```python
from build123d import *


with BuildPart() as part:
    # 草图1 → 旋转1 (revolve)
    with BuildSketch(Plane.XY, mode=Mode.PRIVATE) as revolve_1_sk:
        Polygon((20, 9.76740105), (20, -50.23259895), (51.5, -50.23259895), (51.5, -44.23259895), (57.5, -44.23259895), (57.5, 3.76740105), (51.5, 3.76740105), (51.5, 9.76740105), align=None)
    revolve(revolve_1_sk.sketch.rotate(Axis((0, 27.589183228, 0), (0, -1, 0)), 90), axis=Axis((0, 27.589183228, 0), (0, -1, 0)))


solid = part.part
```
Geometry check sheet. Reference: the model listing, model coordinates, mm. A direction names the side the tool comes from. Round coordinates to 2 decimals unless told otherwise and drop trailing zeros. Order: outer loops, then holes, each group sorted by start corner. A loop starts at its lowest first (then second) coordinate and runs counter-clockwise, first axis right, second up. Notation, with made-up numbers: (58, 56.25) - (77, 56.25) arc R28 cw to (77, 78.25) - close; hole circle Ø8 at (30, 7). An arc over 180 degrees is marked (long way). Use a Markdown table: item, result. Add a question column.
1) Thickness scan on line 1 along X through (y, z) = (-14, 0); line 2 along Y through (x, z) = (-38.5, 38.5); line 3 along Z through (x, y) = (-3, -26). Record the ranges inside material, lowest first.
2) Section check D-D (x = 40.5). Record the cut outline in (y, z), then the cut area to 3 significant figures.
3) Section check A-A (x = 0). Record the cut outline in (y, z).
4) Section check B-B (z = 5). Record the cut outline in (x, y), then the cut area to 3 significant figures.
5) Set-up check for faces 1 (the flat face through (-1, -50.233, -22)), 2 (the flat face through (30, 3.767, -43)): record each of +Z, -Z, +X, -X, +Y, -Y from which the full face is reachable in a straight line by a thin tool's end or side.
6) Mould release check, pull along Z, two halves, no side actions. Record for faces 3 (the cylindrical face through (50.275, -47.191, -11.164)), 4 (the flat face through (30, -44.233, 43)), 5 (the cylindrical face through (-0.88, -20.65, -19.98)): released by +Z, released by -Z, zero draft, split by the parting line, or undercut.
7) Section check C-C (y = -24). Record the cut outline in (x, z), then the cut area to 3 significant figures.
8) Gauge pin test, flat ends, axial feed: P1, Ø5, axis at y = 1.5, z = -5.5, coming from the -X side; P2, Ø2, axis at x = -32, y = -9, coming from the +Z side; P3, Ø5, axis at y = -5, z = -35.5, coming from the -X side. Record the tip position at first contact, or that the pin passes through.
Established:
| question | item | result |
|---|---|---|
| 1 | line 1 | -57.5 to -20, 20 to 57.5 |
| 1 | line 2 | -44.23 to 3.77 |
| 1 | line 3 | -57.42 to -19.77, 19.77 to 57.42 |
| 2 | outline | (-50.23, -31.81) - (-44.23, -31.81) - (-44.23, -40.82) - (3.77, -40.82) - (3.77, -31.81) - (9.77, -31.81) - (9.77, 31.81) - (3.77, 31.81) - (3.77, 40.82) - (-44.23, 40.82) - (-44.23, 31.81) - (-50.23, 31.81) - close |
| 2 | area | 4,680 mm2 |
| 3 | outline | (-50.23, -51.5) - (-44.23, -51.5) - (-44.23, -57.5) - (3.77, -57.5) - (3.77, -51.5) - (9.77, -51.5) - (9.77, -20) - (-50.23, -20) - close; (-50.23, 20) - (9.77, 20) - (9.77, 51.5) - (3.77, 51.5) - (3.77, 57.5) - (-44.23, 57.5) - (-44.23, 51.5) - (-50.23, 51.5) - close |
| 4 | outline | (-57.28, -44.23) - (-51.26, -44.23) - (-51.26, -50.23) - (-19.36, -50.23) - (-19.36, 9.77) - (-51.26, 9.77) - (-51.26, 3.77) - (-57.28, 3.77) - close; (19.36, -50.23) - (51.26, -50.23) - (51.26, -44.23) - (57.28, -44.23) - (57.28, 3.77) - (51.26, 3.77) - (51.26, 9.77) - (19.36, 9.77) - close |
| 4 | area | 4,410 mm2 |
| 5 | face 1 | +Z, -Z, +X, -X, -Y |
| 5 | face 2 | +Y |
| 6 | face 3 | split by the parting line |
| 6 | face 4 | zero draft |
| 6 | face 5 | undercut |
| 7 | outline | circle Ø115 at (0, 0); hole circle Ø40 at (0, 0) |
| 7 | area | 9,130 mm2 |
| 8 | P1 | x = -57.42 |
| 8 | P2 | z = 48.43 |
| 8 | P3 | x = -47.09 |
